Verification items for the finished model (mm, model axes). Coordinates: 2 decimals unless noted, no trailing zeros. Write each loop counter-clockwise with the first axis right and the second up, starting at its lowest first coordinate (ties: lowest second). Pieces come first, ordered by that corner, then holes.
```python
from build123d import *

# Parameters (mm, degrees)
BOSS_EXTRUDE1_DEPTH = 30
FILLET1_R           = 10


with BuildPart() as part:
    # Sketch1 → Boss-Extrude1 (new body)
    with BuildSketch(Plane.XY):
        with BuildLine():
            Line((0, 0), (239, 0))
            Line((239, 0), (239, 840))
            Line((239, 840), (80, 840))
            Line((80, 840), (80, 710))
            ThreePointArc((80, 710), (74.142135624, 695.857864376), (60, 690))
            Line((60, 690), (0, 690))
            Line((0, 690), (0, 0))
        make_face()
    extrude(amount=BOSS_EXTRUDE1_DEPTH)

    # Fillet1
    fillet1_edges = [part.edges().sort_by_distance(p)[0] for p in [
        (239, 840, 15),
    ]]
    fillet(fillet1_edges, radius=FILLET1_R)


solid = part.part
```
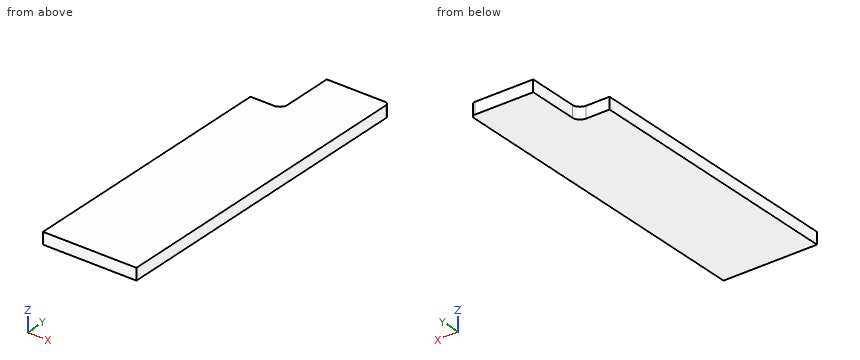
1. Material ranges on L1, parallel to Y at x = 40, z = 22.25; L2, parallel to Y at x = 63, z = 26.25, recorded low to high.
2. Sectioned sample at A-A, the plane z = 24.25. Record the boundary of the cut face in (x, y).
3. Sectioned sample at B-B, the plane x = 42. Record the boundary of the cut face in (y, z), and give its area (3 significant figures).
4. Gauge pin test, flat end, axial feed: P1, Ø15, axis at y = 788, z = 18.5, coming from the -X side. Record the tip position at first contact, or that the pin passes through.
Outcome:
1. L1: y = 0 to 690
1. L2: y = 0 to 690.23
2. outline: (0, 0) - (239, 0) - (239, 830) arc R10 ccw to (229, 840) - (80, 840) - (80, 710) arc R20 cw to (60, 690) - (0, 690) - close
3. outline: (0, 0) - (690, 0) - (690, 30) - (0, 30) - close
3. area: 20,700 mm2
4. P1: stops at x = 80
